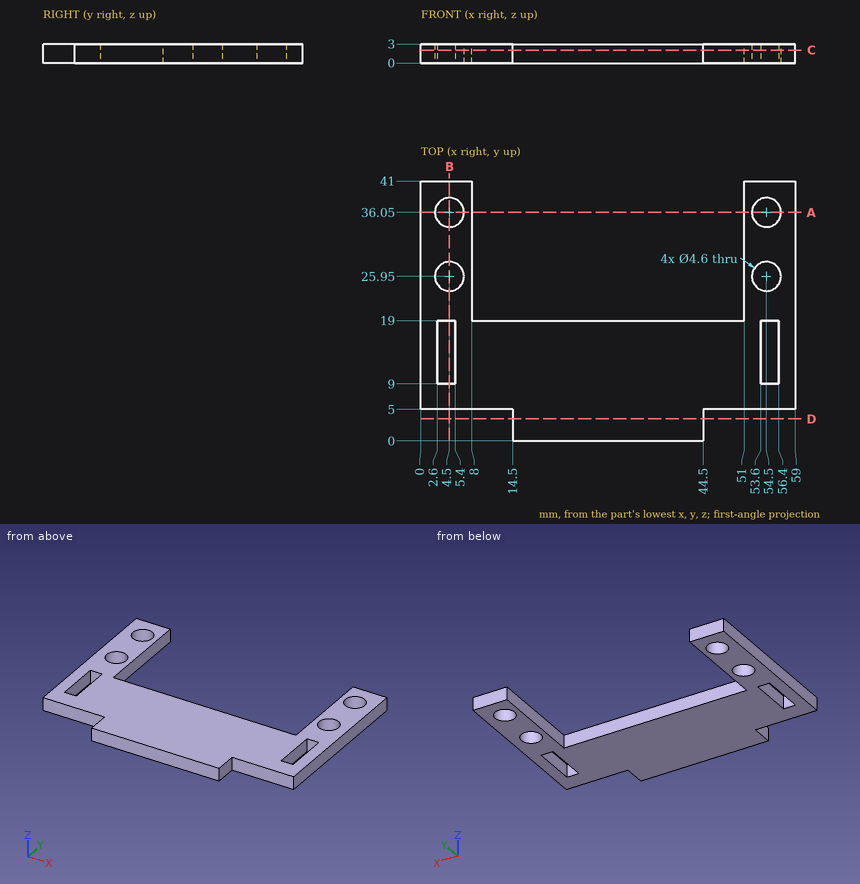
Geometry: see drawing. Coordinates: mm, zero at the bounding-box minimum. Round coordinates to 2 decimals unless told otherwise and drop trailing zeros. Order: outer loops, then holes, each group sorted by start corner. A loop starts at its lowest first (then second) coordinate and runs counter-clockwise, first axis right, second up. Notation, with made-up numbers: (38.5, 75) - (54.5, 75) arc R19 cw to (54.5, 109) - close; hole circle Ø8 at (-26.5, 71). An arc over 180 degrees is marked (long way). Use a Markdown table: item, result. Add a question column.
1. Section query A-A (y = 36.05). Return the cut outline in (x, z).
2. First-contact query: pin 1 (1.5 mm diameter, centred on x = 36.5, z = 1.5, fed in from -Y); pin 2 (1.4 mm diameter, centred on x = 54.5, z = 1, fed in from -Y); pin 3 (4 mm diameter, centred on x = 4.5, y = 36.05, fed in from +Z). Flat tips, straight axial feed; report the tip coordinate or a pass-through.
3. Line query: probe 1 along Y at (x, z) = (4.5, 1.6); probe 2 along X at (y, z) = (14, 1.1); probe 3 along X at (y, z) = (23, 1.2). Output: solid intervals per line, ascending.
4. Section query C-C (z = 2.05). Return the cut outline in (x, y).
5. Section query B-B (x = 4.5). Return the cut outline in (y, z).
6. Section query D-D (y = 3.5). Return the cut outline in (x, z).
Derived:
| question | item | result |
|---|---|---|
| 1 | outline | (0, 0) - (2.2, 0) - (2.2, 3) - (0, 3) - close; (6.8, 0) - (8, 0) - (8, 3) - (6.8, 3) - close; (51, 0) - (52.2, 0) - (52.2, 3) - (51, 3) - close; (56.8, 0) - (59, 0) - (59, 3) - (56.8, 3) - close |
| 2 | pin 1 | y = 0 |
| 2 | pin 2 | y = 5 |
| 2 | pin 3 | through |
| 3 | probe 1 | 5 to 9, 19 to 23.65, 28.25 to 33.75, 38.35 to 41 |
| 3 | probe 2 | 0 to 2.6, 5.4 to 53.6, 56.4 to 59 |
| 3 | probe 3 | 0 to 8, 51 to 59 |
| 4 | outline | (0, 5) - (14.5, 5) - (14.5, 0) - (44.5, 0) - (44.5, 5) - (59, 5) - (59, 41) - (51, 41) - (51, 19) - (8, 19) - (8, 41) - (0, 41) - close; hole circle Ø4.6 at (4.5, 25.95); hole circle Ø4.6 at (4.5, 36.05); hole (2.6, 9) - (5.4, 9) - (5.4, 19) - (2.6, 19) - close; hole circle Ø4.6 at (54.5, 25.95); hole circle Ø4.6 at (54.5, 36.05); hole (53.6, 9) - (56.4, 9) - (56.4, 19) - (53.6, 19) - close |
| 5 | outline | (5, 0) - (9, 0) - (9, 3) - (5, 3) - close; (19, 0) - (23.65, 0) - (23.65, 3) - (19, 3) - close; (28.25, 0) - (33.75, 0) - (33.75, 3) - (28.25, 3) - close; (38.35, 0) - (41, 0) - (41, 3) - (38.35, 3) - close |
| 6 | outline | (14.5, 0) - (44.5, 0) - (44.5, 3) - (14.5, 3) - close |
